Read the model definition and answer for the solid it produces. Units are mm, in the model's axes. A direction names the side the tool comes from. Give positions to 0.01 mm unless a question says otherwise; leave off trailing zeros. Order: outer loops, then holes, each group sorted by start corner. A loop starts at its lowest first (then second) coordinate and runs counter-clockwise, first axis right, second up. Notation, with made-up numbers: (49.25, 48.25) - (100.25, 48.25) arc R24 cw to (100.25, 74.25) - close; hole circle Ø3 at (-36.5, 64). An arc over 180 degrees is marked (long way). Write each question's results on one line, items separated by ' | '. Start each with the question number.
Q1. Find section A-A on z = -1. Give the vertices of the cut face in (x, y), and give its area (3 significant figures).
Q2. Find section D-D on z = -12.5. Give the vertices of the cut face in (x, y), and give its area (3 significant figures).
Q3. Find section B-B on y = 78. Give the vertices of the cut face in (x, z), and give its area (3 significant figures).
Q4. A tool of negligible diameter and unlimited length cuts with its end or side. For faces 4 (the face through (76, 104, 0)), 5 (the face through (39.576, 50.838, 0.28)), 6 (the face through (76, 52, 0)), 7 (the face through (66, 84, -13)), from which of +Z, -Z, +X, -X, +Y, -Y can it reach the whole face along a straight path? Write none if from no direction.
Q5. For a pull along Y with two mould halves and no side action, classify faces 1 (the face through (68, 62, -6)), 2 (the face through (66, 72, -13)), 3 (the face through (16.69, 9.12, 1.08)) as +Y half, -Y half, draft (parallel to the pull), parting line (faces both ways), or undercut.
Q6. Find section C-C on y = 14. Give the vertices of the cut face in (x, z).
Q7. Flat-ended cylindrical pins translate along their axes: P1, Ø6, axis at x = 76, z = 3, coming from the +Y side; P2, Ø20, axis at y = 20.5, z = -7, coming from the -X side; P3, Ø3, axis at y = 66.5, z = -16, coming from the +X side. Find the tip coordinate at first contact, or state that the pin passes through.
Q8. Find the intervals of material crossed by line 1 along X through (y, z) = (26.5, -14.5); line 2 along X through (y, z) = (57.5, -12); line 3 along X through (y, z) = (65.5, -12), in increasing order. Write a range as from..to.
from build123d import *

# Parameters (mm, degrees)
CLAMP_EYE_96X40_DEPTH       = 20
ARM_AND_SMALL_EYE_PROFILE_R = 14
ARM_AND_SMALL_EYE_DEPTH     = 20
CLAMP_SCREW_HOLE_SKETCH_R   = 5
CLAMP_SCREW_HOLE_DEPTH      = 60
ARM_RIB_1_REACH             = 188.473
ARM_RIB_1_SKETCH_WALL_W     = 444.596554162
ARM_RIB_1_SKETCH_WALL_H     = 12
ARM_RIB_2_REACH             = 188.473
ARM_RIB_2_SKETCH_WALL_W     = 444.596554162
ARM_RIB_2_SKETCH_WALL_H     = 12


with BuildPart() as part:
    # Clamp Eye Profile → Clamp Eye Ø96x40 (new, symmetric)
    with BuildSketch(Plane.XY):
        with BuildLine():
            Line((-30, 40.53001201), (-30, 0))
            Line((-30, 0), (-3, 0))
            Line((-3, 0), (-3, 46.140935356))
            ThreePointArc((-3, 46.140935356), (0, 110), (3, 46.140935356))
            Line((3, 46.140935356), (3, 0))
            Line((3, 0), (30, 0))
            Line((30, 0), (30, 40.53001201))
            ThreePointArc((30, 40.53001201), (0, 126), (-30, 40.53001201))
        make_face()
    extrude(amount=CLAMP_EYE_96X40_DEPTH, both=True)

    # Arm and Small Eye Profile → Arm and Small Eye (add, symmetric)
    with BuildSketch(Plane.XY):
        with BuildLine():
            Line((47.623523599, 72), (84.701778719, 72))
            ThreePointArc((84.701778719, 72), (136, 78), (84.701778719, 84))
            Line((84.701778719, 84), (47.623523599, 84))
            ThreePointArc((47.623523599, 84), (48, 78), (47.623523599, 72))
        make_face()
        with Locations((110, 78)):
            Circle(ARM_AND_SMALL_EYE_PROFILE_R, mode=Mode.SUBTRACT)
    extrude(amount=ARM_AND_SMALL_EYE_DEPTH, both=True)

    # Clamp Screw Hole Sketch → Clamp Screw Hole (cut)
    with BuildSketch(Plane(origin=(30, 0, 0), x_dir=(0, 0, -1), z_dir=(1, 0, 0))):
        with Locations((0, 14)):
            Circle(CLAMP_SCREW_HOLE_SKETCH_R)
    extrude(amount=-CLAMP_SCREW_HOLE_DEPTH, mode=Mode.SUBTRACT)

    # Arm Rib 1 Sketch wall → Arm Rib 1 (add, up to next)
    with BuildSketch(Plane(origin=(75.174241002, 104, 0), x_dir=(-1, 0, 0), z_dir=(0, -1, 0)), mode=Mode.PRIVATE) as arm_rib_1_sk1:
        Rectangle(ARM_RIB_1_SKETCH_WALL_W, ARM_RIB_1_SKETCH_WALL_H)
    arm_rib_1_tool1 = extrude(arm_rib_1_sk1.sketch, amount=ARM_RIB_1_REACH, mode=Mode.PRIVATE) - part.part
    add(arm_rib_1_tool1.solids().sort_by_distance((75.174241002, 104, 0))[0])

    # Arm Rib 2 Sketch wall → Arm Rib 2 (add, up to next)
    with BuildSketch(Plane(origin=(75.174241002, 52, 0), x_dir=(-1, 0, 0), z_dir=(0, -1, 0)), mode=Mode.PRIVATE) as arm_rib_2_sk1:
        Rectangle(ARM_RIB_2_SKETCH_WALL_W, ARM_RIB_2_SKETCH_WALL_H)
    arm_rib_2_tool1 = extrude(arm_rib_2_sk1.sketch, amount=-ARM_RIB_2_REACH, mode=Mode.PRIVATE) - part.part
    add(arm_rib_2_tool1.solids().sort_by_distance((75.174241002, 52, 0))[0])


solid = part.part
Working result:
1) outline: (-30, 0) - (-3, 0) - (-3, 9.1) - (-30, 9.1) - close; (-30, 18.9) - (-3, 18.9) - (-3, 46.14) arc R32 cw (long way) to (3, 46.14) - (3, 18.9) - (30, 18.9) - (30, 40.53) arc R48 ccw to (40.35, 52) - (110, 52) arc R26 ccw to (110, 104) - (40.35, 104) arc R48 ccw (long way) to (-30, 40.53) - close; (3, 0) - (30, 0) - (30, 9.1) - (3, 9.1) - close; hole circle Ø28 at (110, 78) | area: 9,010 mm²
2) outline: (-30, 0) - (-3, 0) - (-3, 46.14) arc R32 cw (long way) to (3, 46.14) - (3, 0) - (30, 0) - (30, 40.53) arc R48 ccw to (47.62, 72) - (84.7, 72) arc R26 ccw (long way) to (84.7, 84) - (47.62, 84) arc R48 ccw (long way) to (-30, 40.53) - close; hole circle Ø28 at (110, 78) | area: 7,690 mm²
3) outline: (-48, -20) - (-32, -20) - (-32, 20) - (-48, 20) - close; (32, -20) - (96, -20) - (96, 20) - (32, 20) - close; (124, -20) - (136, -20) - (136, 20) - (124, 20) - close | area: 3,680 mm²
4) face 4: +Z, -Z, +X, +Y | face 5: -Y | face 6: +Z, -Z, +X, -Y | face 7: -Z, +Y
5) face 1: draft | face 2: -Y half | face 3: undercut
6) outline: (-30, -20) - (-3, -20) - (-3, -5) - (-30, -5) - close; (-30, 5) - (-3, 5) - (-3, 20) - (-30, 20) - close; (3, -20) - (30, -20) - (30, -5) - (3, -5) - close; (3, 5) - (30, 5) - (30, 20) - (3, 20) - close
7) P1: y = 104 | P2: x = -30 | P3: x = 134
8) line 1: -30..-3, 3..30 | line 2: -43.4..-24.57, 24.57..43.4, 94.01..125.99 | line 3: -46.34..-29.46, 29.46..46.34, 87.2..103.7, 116.3..132.8
